```python
from build123d import *

# Parameters (mm, degrees)
SKETCH1_W             = 12
SKETCH1_H             = 3
BOSS_EXTRUDE1_DEPTH   = 840
SKETCH2_W             = 10
SKETCH2_H             = 1
CUT_EXTRUDE1_DEPTH    = 841.951655259
M6_TAPPED_HOLE1_D     = 5
M6_TAPPED_HOLE1_DEPTH = 15
M6_TAPPED_HOLE1_TIP   = 1.502151548


with BuildPart() as part:
    # Sketch1 → Boss-Extrude1 (new body)
    with BuildSketch(Plane.XY):
        with Locations((-25.901003365, 22.624934563)):
            Rectangle(SKETCH1_W, SKETCH1_H)
    extrude(amount=BOSS_EXTRUDE1_DEPTH)

    # Sketch2 → Cut-Extrude1 (cut, through all)
    with BuildSketch(Plane.XY.offset(840)):
        with Locations((-25.901003365, 22.624934563)):
            Rectangle(SKETCH2_W, SKETCH2_H)
    extrude(amount=-CUT_EXTRUDE1_DEPTH, mode=Mode.SUBTRACT)

    # M6 Tapped Hole1
    with Locations(Plane(origin=(-25.901003365, 24.124934563, 389), x_dir=(0, 0, 1), z_dir=(0, 1, 0))):
        with Locations((0, 0), (62, 0)):
            Hole(M6_TAPPED_HOLE1_D / 2, depth=M6_TAPPED_HOLE1_DEPTH)
            with Locations((0, 0, -(M6_TAPPED_HOLE1_DEPTH + M6_TAPPED_HOLE1_TIP / 2))):  # 118° drill point
                Cone(0, M6_TAPPED_HOLE1_D / 2, M6_TAPPED_HOLE1_TIP, mode=Mode.SUBTRACT)


solid = part.part
```
Check sheet for the modelled part. Datum: model origin and axes. Units: mm. Round coordinates to 2 decimals unless told otherwise and drop trailing zeros. Order: outer loops, then holes, each group sorted by start corner. A loop starts at its lowest first (then second) coordinate and runs counter-clockwise, first axis right, second up. Notation, with made-up numbers: M 12,62.25 L 70,62.25 A24 cw 70,91.25 Z; hole C 55.5,62.5 d7. An arc over 180 degrees is marked long. Answer in a Markdown table with one row per item.
(1) Section check A-A on z = 485. Record the boundary of the cut face in (x, y), plus the area to 3 significant figures.
Findings:
| item | result |
|---|---|
| outline | M -31.9,21.12 L -19.9,21.12 L -19.9,24.12 L -31.9,24.12 Z; hole M -30.9,22.12 L -20.9,22.12 L -20.9,23.12 L -30.9,23.12 Z |
| area | 26.0 mm^2 |
(2) Gauge pin test, flat ends, axial feed: pin 1 (3 mm diameter, centred on x = -25.9, z = 389, fed in from +Y); pin 2 (6.5 mm diameter, centred on x = -25.9, z = 451, fed in from +Y). Record the tip position at first contact, or that the pin passes through.
Findings:
| item | result |
|---|---|
| pin 1 | passes through |
| pin 2 | stops at y = 24.12 |
(3) Material ranges on line 1 along Y through (x, z) = (-24.75, 139); line 2 along Z through (x, y) = (-24.75, 23.2); line 3 along X through (y, z) = (22.65, 400.5), recorded low to high. Write a range as from..to.
Findings:
| item | result |
|---|---|
| line 1 | y = 21.12..22.12, 23.12..24.12 |
| line 2 | z = 0..386.78, 391.22..448.78, 453.22..840 |
| line 3 | x = -31.9..-30.9, -20.9..-19.9 |
(4) Section check B-B on y = 22.6. Record the boundary of the cut face in (x, z).
Findings:
| item | result |
|---|---|
| outline | M -31.9,0 L -30.9,0 L -30.9,840 L -31.9,840 Z; M -20.9,0 L -19.9,0 L -19.9,840 L -20.9,840 Z |
